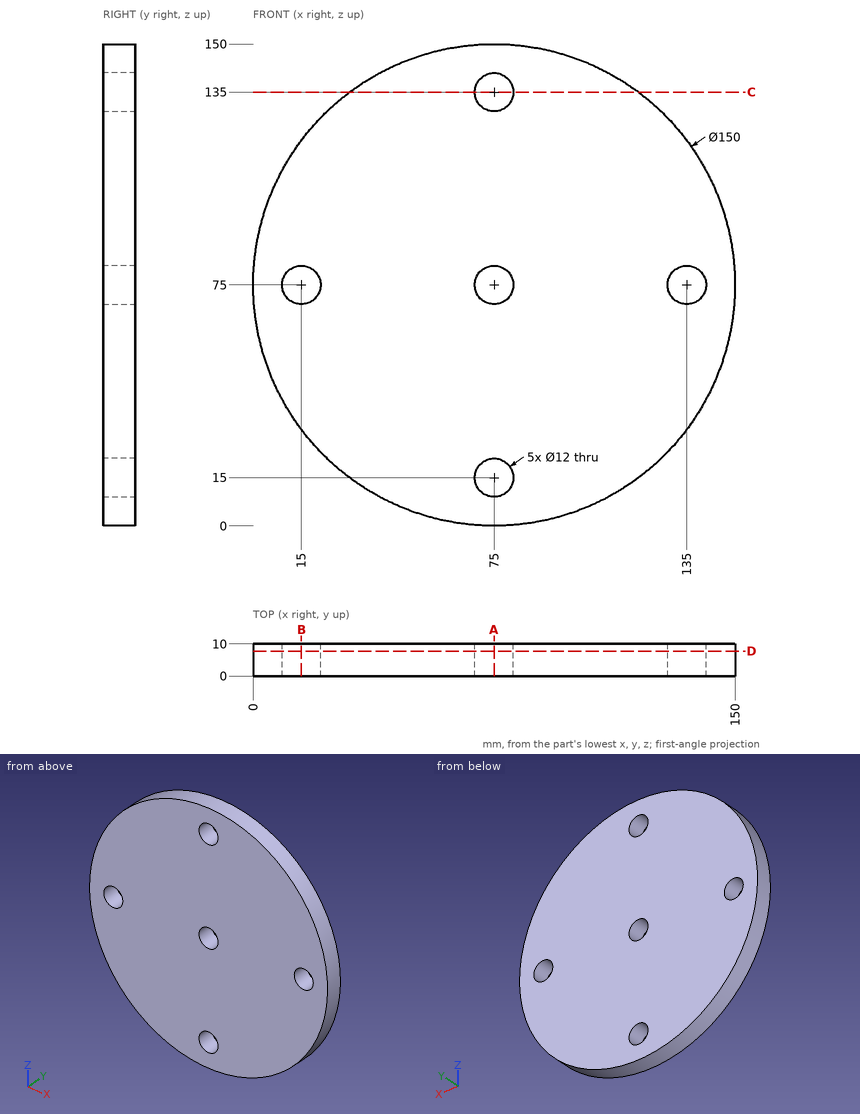
The figure shows three views and two pictorial views of one solid part (mm, origin at its lowest corner). Answer the questions. Coordinates: 2 decimals unless noted, no trailing zeros. Write each loop counter-clockwise with the first axis right and the second up, starting at its lowest first coordinate (ties: lowest second). Pieces come first, ordered by that corner, then holes. Notation, with made-up numbers: (-19.5, 34.25) -> (-7.5, 34.25) arc R16 ccw to (-7.5, 45.25) -> close; hole circle Ø2 at (63.5, -34). An arc over 180 degrees is marked (long way). Return JSON: item names as keys, results as strings.
(1) The part is cut by section D-D on y = 7.75. Give the vertices of the cut face in (x, z).
Answers below:
{"outline": "circle Ø150 at (75, 75); hole circle Ø12 at (15, 75); hole circle Ø12 at (75, 15); hole circle Ø12 at (75, 75); hole circle Ø12 at (75, 135); hole circle Ø12 at (135, 75)"}
(2) Consider line 1 along X through (y, z) = (5, 75); line 2 along X through (y, z) = (6, 135); line 3 along Z through (x, y) = (136.5, 2.5). Determine where each line is inside the solid, lowest interval first. Write a range as from..to.
Answers below:
{"line 1": "0..9, 21..69, 81..129, 141..150", "line 2": "30..69, 81..120", "line 3": "32.07..69.19, 80.81..117.93"}
(3) Each of these flat-tipped pins is pushed along its axis until it touches: P1, Ø4, axis at x = 26, y = 2.5, coming from the -Z side; P2, Ø4, axis at y = 6, z = 83.5, coming from the +X side; P3, Ø2, axis at x = 15.5, y = 6.5, coming from the +Z side. Where does it stop, or does it pass through?
Answers below:
{"P1": "z = 16.55", "P2": "x = 149.72", "P3": "z = 121.93"}
(4) The part is cut by section B-B on x = 15. Give the vertices of the cut face in (y, z).
Answers below:
{"outline": "(0, 30) -> (10, 30) -> (10, 69) -> (0, 69) -> close; (0, 81) -> (10, 81) -> (10, 120) -> (0, 120) -> close"}
(5) The part is cut by section A-A on x = 75. Give the vertices of the cut face in (y, z), then the cut area to 3 significant figures.
Answers below:
{"outline": "(0, 0) -> (10, 0) -> (10, 9) -> (0, 9) -> close; (0, 21) -> (10, 21) -> (10, 69) -> (0, 69) -> close; (0, 81) -> (10, 81) -> (10, 129) -> (0, 129) -> close; (0, 141) -> (10, 141) -> (10, 150) -> (0, 150) -> close", "area": "1,140 mm^2"}
(6) The part is cut by section C-C on z = 135. Give the vertices of the cut face in (x, y).
Answers below:
{"outline": "(30, 0) -> (69, 0) -> (69, 10) -> (30, 10) -> close; (81, 0) -> (120, 0) -> (120, 10) -> (81, 10) -> close"}
